```python
from build123d import *

# Parameters (mm, degrees)
BASE_EXTRUDE_DEPTH      = 0.75
BASE_EXTRUDE_DEPTH_BACK = 0.75
SKETCH1_R               = 1.25


with BuildPart() as part:
    # Sketch1 → Base-Extrude (new, two sides: drawn at the far end of the back side and taken through both)
    with BuildSketch(Plane.XY.offset(-BASE_EXTRUDE_DEPTH_BACK)):
        with BuildLine():
            Line((-1.5, -17.159971928), (-1.5, -22.778094604))
            ThreePointArc((-1.5, -22.778094604), (-5.452894614, -22.133712537), (-9.220039428, -20.773850767))
            ThreePointArc((-9.220039428, -20.773850767), (-9.404653614, -20.625111252), (-9.5, -20.408051566))
            Line((-9.5, -20.408051566), (-10.086937259, -17.079364962))
            ThreePointArc((-10.086937259, -17.079364962), (-10.239358111, -16.698818185), (-10.531659889, -16.411402743))
            ThreePointArc((-10.531659889, -16.411402743), (0, 19.5), (10.531659889, -16.411402743))
            ThreePointArc((10.531659889, -16.411402743), (10.239358111, -16.698818185), (10.086937259, -17.079364962))
            Line((10.086937259, -17.079364962), (9.5, -20.408051566))
            ThreePointArc((9.5, -20.408051566), (9.404653614, -20.625111252), (9.220039428, -20.773850767))
            ThreePointArc((9.220039428, -20.773850767), (5.452894614, -22.133712537), (1.5, -22.778094604))
            Line((1.5, -22.778094604), (1.5, -17.159971928))
            ThreePointArc((1.5, -17.159971928), (0, 14.97), (-1.5, -17.159971928))
        make_face()
        with Locations((-5.5, -19.212035284)):
            Circle(SKETCH1_R, mode=Mode.SUBTRACT)
        with Locations(Location((5.5, -19.212035284, 0), (0, 0, 180))):
            Circle(SKETCH1_R, mode=Mode.SUBTRACT)
    extrude(amount=BASE_EXTRUDE_DEPTH + BASE_EXTRUDE_DEPTH_BACK)


solid = part.part
```
Source: CAD feature listing. Evaluate the final solid. Frame: model axes, mm. A direction names the side the tool comes from. Give positions to 0.01 mm unless a question says otherwise; leave off trailing zeros. Loops run counter-clockwise (first coordinate to the right, second up) from the corner with the lowest first, then second, coordinate; pieces in that order, holes last. Notation, with made-up numbers: (-35.75, -24.75) -> (7.25, -24.75) arc R20 cw to (7.25, -1.75) -> close; hole circle Ø7 at (73, 58). An arc over 180 degrees is marked (long way). Put each result on its own line as item: value. Start each with the question number.
1) Reachability of faces 5 (the face through (-1.5, -20, 0)), 6 (the face through (-9.79, -18.77, -0.01)) from +Z, -Z, +X, -X, +Y, -Y: full face, straight path, thin tool, end or side. Return the list, or none.
2) Cut plane C-C (z = -0.35). Return loops of the section in (x, y), then the cut area to 3 significant figures.
3) Draft query along Y for faces 1 (the face through (5.8, -18, 0)), 2 (the face through (-0.702, 19.487, -0.01)), 3 (the face through (1.5, -20, 0)), 4 (the face through (9.8, -18.7, 0)). Return one class per face: released by +Y, released by -Y, zero draft, split by the parting line, or undercut.
4) Cut plane A-A (y = 6). Return loops of the section in (x, z).
5) Material intervals for probe 1 along Y at (x, z) = (-5.5, 0.05); probe 2 along X at (y, z) = (-7, -0.45); probe 3 along X at (y, z) = (-1.13, 0.1), sorted ascending.
6) Cut plane D-D (x = 0). Return loops of the section in (y, z), then the cut area to 4 significant figures.
7) Contact query for flat-ended pins moving along their axis: P1, Ø0.8, axis at y = -20, z = 0, coming from the +X side; P2, Ø10, axis at x = 8, y = -11.5, coming from the +Z side. Output: stop coordinate, or through.
8) Cut plane B-B (x = -8.5). Return loops of the section in (y, z).
Results are:
1. face 5: +Z, -Z, -Y
1. face 6: +Z, -Z, -X, -Y
2. outline: (-10.53, -16.41) arc R1 cw to (-10.09, -17.08) -> (-9.5, -20.41) arc R0.5 ccw to (-9.22, -20.77) arc R21.7 ccw to (-1.5, -22.78) -> (-1.5, -17.16) arc R16.1 cw (long way) to (1.5, -17.16) -> (1.5, -22.78) arc R21.7 ccw to (9.22, -20.77) arc R0.5 ccw to (9.5, -20.41) -> (10.09, -17.08) arc R1 cw to (10.53, -16.41) arc R19.5 ccw (long way) to start; hole circle Ø2.5 at (-5.5, -19.21); hole circle Ø2.5 at (5.5, -19.21)
2. area: 421 mm2
3. face 1: undercut
3. face 2: split by the parting line
3. face 3: zero draft
3. face 4: released by -Y
4. outline: (-18.55, -0.75) -> (-14.44, -0.75) -> (-14.44, 0.75) -> (-18.55, 0.75) -> close; (14.44, -0.75) -> (18.55, -0.75) -> (18.55, 0.75) -> (14.44, 0.75) -> close
5. probe 1: y = -22.12 to -20.46, -17.96 to -16.26, 14 to 18.71
5. probe 2: x = -18.2 to -14.99, 14.99 to 18.2
5. probe 3: x = -19.47 to -16.1, 16.1 to 19.47
6. outline: (14.97, -0.75) -> (19.5, -0.75) -> (19.5, 0.75) -> (14.97, 0.75) -> close
6. area: 6.795 mm2
7. P1: stops at x = 9.64
7. P2: stops at z = 0.75
8. outline: (-21.1, -0.75) -> (-14.8, -0.75) -> (-14.8, 0.75) -> (-21.1, 0.75) -> close; (12.54, -0.75) -> (17.55, -0.75) -> (17.55, 0.75) -> (12.54, 0.75) -> close
